```python
from build123d import *

# Parameters (mm, degrees)
SKETCH_2_R             = 17.5
CUT_EXTRUDE_1_DEPTH    = 169.650526237
HOLE_WIZARD_M6_1_D     = 6.6
HOLE_WIZARD_M8_1_D     = 6.8
HOLE_WIZARD_M8_1_DEPTH = 19.75
HOLE_WIZARD_M8_1_TIP   = 2.042926105
SKETCH_9_W             = 15
SKETCH_9_H             = 23


with BuildPart() as part:
    # 草图1 → 旋转1 (revolve)
    with BuildSketch(Plane.XY, mode=Mode.PRIVATE) as revolve_1_sk:
        Polygon((0, 0), (70, 0), (70, 6), (91, 6), (91, 58), (50, 58), (50, 88), (25, 88), (25, 97), (20.5, 97), (20.5, 109), (0, 109), align=None)
    revolve(revolve_1_sk.sketch.rotate(Axis((0, 0, 0), (0, 1, 0)), 90), axis=Axis((0, 0, 0), (0, 1, 0)))

    # 草图2 → 切除-拉伸1 (cut, through all)
    with BuildSketch(Plane(origin=(0, 109, 0), x_dir=(1, 0, 0), z_dir=(0, 1, 0))):
        with Locations(Location((0, 0, 0), (0, 0, 270))):
            Circle(SKETCH_2_R)
    extrude(amount=-CUT_EXTRUDE_1_DEPTH, mode=Mode.SUBTRACT)

    # M6 间隙孔1 (through all)
    with Locations(Plane(origin=(0, 58, 0), x_dir=(1, 0, 0), z_dir=(0, 1, 0))):
        with Locations((0, 84), (42, 72.746133918), (72.746133918, 42), (84, 0), (72.746133918, -42), (42, -72.746133918), (0, -84), (-42, -72.746133918), (-72.746133918, -42), (-84, 0), (-72.746133918, 42), (-42, 72.746133918)):
            Hole(HOLE_WIZARD_M6_1_D / 2)

    # M8 螺纹孔1
    with Locations(Plane(origin=(0, 0, 0), x_dir=(-1, 0, 0), z_dir=(0, -1, 0))):
        with Locations((0, 58), (41.012193309, 41.012193309), (58, 0), (41.012193309, -41.012193309), (0, -58), (-41.012193309, -41.012193309), (-58, 0), (-41.012193309, 41.012193309)):
            Hole(HOLE_WIZARD_M8_1_D / 2, depth=HOLE_WIZARD_M8_1_DEPTH)
            with Locations((0, 0, -(HOLE_WIZARD_M8_1_DEPTH + HOLE_WIZARD_M8_1_TIP / 2))):  # 118° drill point
                Cone(0, HOLE_WIZARD_M8_1_D / 2, HOLE_WIZARD_M8_1_TIP, mode=Mode.SUBTRACT)

    # 草图9 → 切除-旋转1 (revolve, cut)
    with BuildSketch(Plane.XY, mode=Mode.PRIVATE) as cut_revolve_1_sk:
        with Locations((42.5, 69.5)):
            Rectangle(SKETCH_9_W, SKETCH_9_H)
    revolve(cut_revolve_1_sk.sketch.rotate(Axis((0, 0, 0), (0, -1, 0)), 270), axis=Axis((0, 0, 0), (0, -1, 0)), mode=Mode.SUBTRACT)


solid = part.part
```
Work out the finished part from the listing and answer in its coordinate system (mm). A direction names the side the tool comes from. Give positions to 0.01 mm unless a question says otherwise; leave off trailing zeros. Loops run counter-clockwise (first coordinate to the right, second up) from the corner with the lowest first, then second, coordinate; pieces in that order, holes last. Notation, with made-up numbers: M 80.5,-19.75 L 118.5,-19.75 A18 ccw 118.5,8.25 Z; hole C 72,89.5 d7. An arc over 180 degrees is marked long. One line per item, written item: value. Start each with the question number.
1. Find section D-D (x = 72.5). Give the vertices of the cut face in (y, z).
2. Find section C-C (y = 53). State how many separate pieces and enclosed holes the cut face has, and give its area (3 significant figures).
3. Each of these flat-tipped pins is pushed along its axis until it touches: P1, Ø10, axis at x = 64, z = -30.5, coming from the +Y side; P2, Ø1, axis at y = 19, z = 26, coming from the +X side; P3, Ø1.5, axis at y = 46, z = -72.5, coming from the -X side. Where does it stop, or does it pass through?
4. Find the intervals of material crossed by probe 1 along X at (y, z) = (32.5, -42); probe 2 along Y at (x, z) = (-5.5, 40.5); probe 3 along Z at (x, y) = (84, 27), in increasing order.
5. Which of the six approach directions +Z, -Z, +X, -X, +Y, -Y give full straight-line access (tool end or side, diameter ignored) to faces 5 (the face through (76.043, 31.636, -42.145)), 6 (the face through (37.615, 10.013, -41.162)), 7 (the face through (-1, 58, -39)), 8 (the face through (-7.509, 92.563, -23.846))?
6. Determine the mould class of faces 1 (the face through (-58.27, 21.44, 0.52)), 2 (the face through (15, 0, 15)), 3 (the face through (7.852, 103.084, -18.937)), 4 (the face through (0.077, 21.438, -58.585)) for opening direction X: released by +X, released by -X, zero draft, split by the parting line, or undercut.
7. Find section B-B (z = -84). Give the vertices of the cut face in (x, y).
8. Find section A-A (x = -84). Give the vertices of the cut face in (y, z).
Reported:
1. outline: M 6,-55 L 58,-55 L 58,-45.29 L 6,-45.29 Z; M 6,-38.71 L 58,-38.71 L 58,38.71 L 6,38.71 Z; M 6,45.29 L 58,45.29 L 58,55 L 6,55 Z
2. separate pieces: 1
2. enclosed holes: 13
2. area: 24,600 mm²
3. P1: stops at y = 58
3. P2: stops at x = 87.35
3. P3: stops at x = -55.97
4. probe 1: x = -80.73 to -76.05, -69.45 to 69.45, 76.05 to 80.73
4. probe 2: y = 0 to 58, 81 to 88
4. probe 3: z = -35 to -3.3, 3.3 to 35
5. face 5: +Y, -Y
5. face 6: -Y
5. face 7: none
5. face 8: +Y
6. face 1: undercut
6. face 2: zero draft
6. face 3: split by the parting line
6. face 4: undercut
7. outline: M -35,6 L -3.3,6 L -3.3,58 L -35,58 Z; M 3.3,6 L 35,6 L 35,58 L 3.3,58 Z
8. outline: M 6,-35 L 58,-35 L 58,-3.3 L 6,-3.3 Z; M 6,3.3 L 58,3.3 L 58,35 L 6,35 Z
